from build123d import *

# Parameters (mm, degrees)
SKETCH_1_W                = 20
SKETCH_1_H                = 17.5
EXTRUDE_1_DEPTH           = 1630
HOLE_WIZARD_1_D           = 5.5
HOLE_WIZARD_1_CBORE_D     = 10
HOLE_WIZARD_1_CBORE_DEPTH = 5.7
PATTERN_LINEAR_1_COUNT    = 27
PATTERN_LINEAR_1_PITCH    = 60


with BuildPart() as part:
    # 草图1 → 凸台-拉伸1 (new body)
    with BuildSketch(Plane.XY):
        with Locations((10, 8.75)):
            Rectangle(SKETCH_1_W, SKETCH_1_H)
    extrude(amount=EXTRUDE_1_DEPTH)

    # 打孔尺寸(%根据)内六角圆柱头螺钉的类型1 (through all)
    with Locations(Plane(origin=(0, 0, 0), x_dir=(-1, 0, 0), z_dir=(0, -1, 0))):
        with Locations((-10, -1600)):
            hole_wizard_1 = CounterBoreHole(HOLE_WIZARD_1_D / 2, HOLE_WIZARD_1_CBORE_D / 2, HOLE_WIZARD_1_CBORE_DEPTH)

    # 阵列(线性)1: 打孔尺寸(%根据)内六角圆柱头螺钉的类型1 ×27
    with Locations(*[(0, 0, -i * PATTERN_LINEAR_1_PITCH) for i in range(1, PATTERN_LINEAR_1_COUNT)]):
        add(hole_wizard_1, mode=Mode.SUBTRACT)


solid = part.part
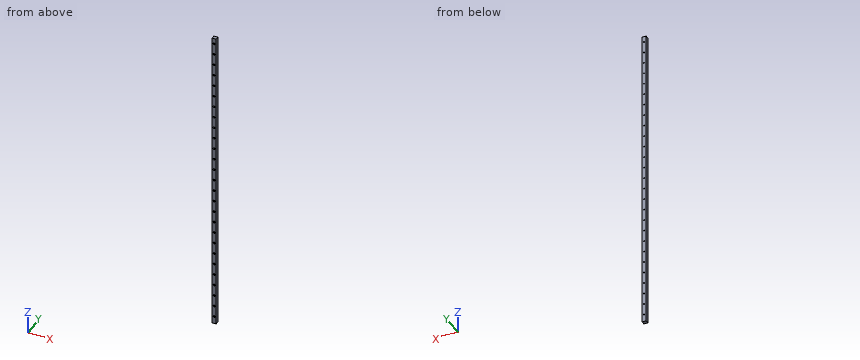
Read the model definition and answer for the solid it produces. Units are mm, in the model's axes. Give positions to 0.01 mm unless a question says otherwise; leave off trailing zeros. Use CSV: the item, a comma, the result in double quotes. Start each with the question number.
(1) Given P1, Ø5, axis at x = 10, z = 221, coming from the -Y side; P2, Ø4.5, axis at x = 10, z = 880, coming from the -Y side, each flat-ended and moving along its own axis, determine where each tip first touches the part or whether it passes through.
(2) Find section A-A (y = 11). Count the separate pieces of the cut face and the enclosed holes in it, plus the area to 3 significant figures.
(3) Consider line 1 along X through (y, z) = (1.8, 880); line 2 along X through (y, z) = (10.75, 1240). Determine where each line is inside the solid, lowest interval first.
Findings below:
1,P1,"y = 5.7"
1,P2,"through"
2,separate pieces,"1"
2,enclosed holes,"27"
2,area,"32,000 mm2"
3,line 1,"0 to 5, 15 to 20"
3,line 2,"0 to 7.25, 12.75 to 20"
